```python
from build123d import *

# Parameters (mm, degrees)
EXTRUDE_1_DEPTH        = 50
CHAMFER_1_SIZE         = 0.7
PATTERN_LINEAR_1_COUNT = 2
PATTERN_LINEAR_1_PITCH = 60
MOVE_FACE_1_BY         = 10
MOVE_FACE_2_BY         = 10


with BuildPart() as part:
    # 草图1 → 凸台-拉伸1 (new, symmetric)
    with BuildSketch(Plane.XY):
        Polygon((-7.5, 0), (7.5, 0), (7.5, 4.3), (6.375, 5.425), (6.375, 9.65), (7.5, 10.775), (7.5, 15), (-7.5, 15), (-7.5, 10.775), (-6.375, 9.65), (-6.375, 5.425), (-7.5, 4.3), align=None)
    extrude(amount=EXTRUDE_1_DEPTH, both=True)

    # 倒角1
    chamfer_1_edges = [part.edges().sort_by_distance(p)[0] for p in [
        (7.5, 0, 0),
        (-7.5, 0, 0),
    ]]
    chamfer(chamfer_1_edges, length=CHAMFER_1_SIZE)

    # 草图3 → Cut-Revolve 1095 (revolve, cut)
    with BuildSketch(Plane(origin=(0, 0, 0), x_dir=(0, 0, -1), z_dir=(1, 0, 0)), mode=Mode.PRIVATE) as cut_revolve_1095_sk:
        Polygon((-30, 15), (-33.75, 15), (-33.75, 9.7), (-32.25, 9.7), (-32.25, 0), (-30, 0), align=None)
    cut_revolve_1095 = revolve(cut_revolve_1095_sk.sketch.rotate(Axis((0, 15, 30), (0, 1, 0)), 180), axis=Axis((0, 15, 30), (0, 1, 0)), mode=Mode.SUBTRACT)

    # 上锁孔阵列(线性)1: Cut-Revolve 1095 ×2
    with Locations(*[(0, 0, -i * PATTERN_LINEAR_1_PITCH) for i in range(1, PATTERN_LINEAR_1_COUNT)]):
        add(cut_revolve_1095, mode=Mode.SUBTRACT)

    # Move Face 1: a face moved outward by 10.0
    extrude(part.faces().sort_by_distance((0, 7.514633707, 50))[0], amount=MOVE_FACE_1_BY, dir=(0, 0, 1))

    # Move Face 2: a face moved outward by 10.0
    extrude(part.faces().sort_by_distance((0, 7.514633707, -50))[0], amount=MOVE_FACE_2_BY, dir=(0, 0, -1))


solid = part.part
```
The model under review builds one solid part; all positions refer to its coordinate system, in mm. A direction names the side the tool comes from. Coordinates: 2 decimals unless noted, no trailing zeros. Write each loop counter-clockwise with the first axis right and the second up, starting at its lowest first coordinate (ties: lowest second). Pieces come first, ordered by that corner, then holes. Notation, with made-up numbers: (76.25, 12.5) - (134.25, 12.5) arc R17 ccw to (134.25, 21.5) - close; hole circle Ø10 at (-9, 72.25). An arc over 180 degrees is marked (long way). Write item = value, one per line.
(1) For P1, Ø2.5, axis at x = 0, z = 30, coming from the -Y side; P2, Ø6, axis at x = 0, z = -30, coming from the +Y side; P3, Ø1.3, axis at y = 8, z = 24, coming from the -X side (3 decimals); P4, Ø2, axis at y = 8, z = -15.5, coming from the +X side (3 decimals), all flat-tipped, find the tip position at first contact; note any pin that passes through.
Result sheet:
P1 = through
P2 = 9.7
P3 = -6.375
P4 = 6.375
(2) Consider section B-B, the plane x = 0. Give the boundary of the cut face in (y, z), then the cut area to 3 significant figures.
Result sheet:
outline = (0, -60) - (15, -60) - (15, -33.75) - (9.7, -33.75) - (9.7, -32.25) - (0, -32.25) - close; (0, -27.75) - (9.7, -27.75) - (9.7, -26.25) - (15, -26.25) - (15, 26.25) - (9.7, 26.25) - (9.7, 27.75) - (0, 27.75) - close; (0, 32.25) - (9.7, 32.25) - (9.7, 33.75) - (15, 33.75) - (15, 60) - (0, 60) - close
area = 1,630 mm^2
(3) Consider section C-C, the plane y = 13.75. Give the boundary of the cut face in (x, z), then the cut area to 3 significant figures.
Result sheet:
outline = (-7.5, -60) - (7.5, -60) - (7.5, 60) - (-7.5, 60) - close; hole circle Ø7.5 at (0, -30); hole circle Ø7.5 at (0, 30)
area = 1,710 mm^2
(4) Consider section D-D, the plane z = 16. Give the boundary of the cut face in (x, y) (3 decimals), then the cut area to 3 significant figures.
Result sheet:
outline = (-7.5, 0.7) - (-6.8, 0) - (6.8, 0) - (7.5, 0.7) - (7.5, 4.3) - (6.375, 5.425) - (6.375, 9.65) - (7.5, 10.775) - (7.5, 15) - (-7.5, 15) - (-7.5, 10.775) - (-6.375, 9.65) - (-6.375, 5.425) - (-7.5, 4.3) - close
area = 212 mm^2
(5) Consider section A-A, the plane z = 30. Give the boundary of the cut face in (x, y) (3 decimals), then the cut area to 3 significant figures.
Result sheet:
outline = (-7.5, 0.7) - (-6.8, 0) - (-2.25, 0) - (-2.25, 9.7) - (-3.75, 9.7) - (-3.75, 15) - (-7.5, 15) - (-7.5, 10.775) - (-6.375, 9.65) - (-6.375, 5.425) - (-7.5, 4.3) - close; (2.25, 0) - (6.8, 0) - (7.5, 0.7) - (7.5, 4.3) - (6.375, 5.425) - (6.375, 9.65) - (7.5, 10.775) - (7.5, 15) - (3.75, 15) - (3.75, 9.7) - (2.25, 9.7) - close
area = 129 mm^2
(6) Machinability: for faces 5 (the face through (0, 8, 60)), 6 (the face through (0, 15, 1)), 7 (the face through (-2.534, 12.313, 32.764)), 8 (the face through (-6.375, 8, 1)), 9 (the face through (6.375, 8, 1)), which of the approach directions +Z, -Z, +X, -X, +Y, -Y give a long, thin tool a straight path to every point of the face, cutting with its end or side? Answer none if there is none.
Result sheet:
face_5 = +Z, +X, -X, +Y, -Y
face_6 = +Z, -Z, +X, -X, +Y
face_7 = +Y
face_8 = +Z, -Z, -X
face_9 = +Z, -Z, +X
(7) Mouldability with a two-part tool opening along Z and no side actions: class faces 1 (the face through (2, 9.7, -32)), 2 (the face through (0.86, 4.78, -32.08)), 3 (the face through (0, 0, 1)), 4 (the face through (0, 8, -60)) as pulls with the +Z half, pulls with the -Z half, needs draft (parallel to the pull), parting line crosses it, or undercut.
Result sheet:
face_1 = undercut
face_2 = undercut
face_3 = needs draft
face_4 = pulls with the -Z half
(8) For line 1 (X direction, y = 13.35, z = -30); line 2 (Z direction, x = 1, y = 5); line 3 (Y direction, x = 0.5, z = -27.5), list the stretches that pass through material, from the lowest coordinate up. Write a range as [from, to].
Result sheet:
line_1 = [-7.5, -3.75], [3.75, 7.5]
line_2 = [-60, -32.02], [-27.98, 27.98], [32.02, 60]
line_3 = [0, 9.7]
